The listing builds one solid part. Answer for the finished solid, in the listing's coordinates (mm). A direction names the side the tool comes from. Give positions to 0.01 mm unless a question says otherwise; leave off trailing zeros. Loops run counter-clockwise (first coordinate to the right, second up) from the corner with the lowest first, then second, coordinate; pieces in that order, holes last. Notation, with made-up numbers: (57.5, 76.5) - (101.5, 76.5) arc R30 ccw to (101.5, 99.5) - close; hole circle Ø10 at (-26.75, 42.5). An arc over 180 degrees is marked (long way). Write each question's results on one line, items separated by ' | '.
from build123d import *

# Parameters (mm, degrees)
SKETCH1_R           = 8
SKETCH1_R_2         = 8.25
BOSS_EXTRUDE1_DEPTH = 426


with BuildPart() as part:
    # Sketch1 → Boss-Extrude1 (new body)
    with BuildSketch(Plane.XY):
        with BuildLine():
            Line((-189.997809191, -121.602817484), (-189.997809191, -92.231705942))
            ThreePointArc((-189.997809191, -92.231705942), (-108.380706485, 81.229274354), (-36.431596452, -96.459748112))
            Line((-36.431596452, -96.459748112), (-40.758896177, -121.602817484))
            Line((-40.758896177, -121.602817484), (42.120800042, -121.602817484))
            ThreePointArc((42.120800042, -121.602817484), (-111.259960397, 158.805233349), (-264.640720837, -121.602817484))
            Line((-264.640720837, -121.602817484), (-189.997809191, -121.602817484))
        make_face()
        with Locations((-24.992933093, 62.919265507)):
            Circle(SKETCH1_R, mode=Mode.SUBTRACT)
        with Locations((-197.526987702, 62.919265507)):
            Circle(SKETCH1_R, mode=Mode.SUBTRACT)
        with Locations((-210.852881833, -80.847761798)):
            Circle(SKETCH1_R_2, mode=Mode.SUBTRACT)
        with Locations((-11.667038962, -80.847761798)):
            Circle(SKETCH1_R_2, mode=Mode.SUBTRACT)
    extrude(amount=-BOSS_EXTRUDE1_DEPTH)


solid = part.part
Item 1: Flat-ended cylindrical pins translate along their axes: P1, Ø8, axis at y = 103.5, z = -118.5, coming from the -X side; P2, Ø6, axis at y = -77, z = -167, coming from the -X side; P3, Ø10, axis at y = 96.5, z = -44, coming from the -X side; P4, Ø13, axis at x = -11.67, y = -80.85, coming from the +Z side. Find the tip coordinate at first contact, or state that the pin passes through.
Values found:
P1: stops at x = -245.75 | P2: stops at x = -286.23 | P3: stops at x = -252.64 | P4: passes through
Item 2: For a pull along Y with two mould halves and no side action, classify faces 4 (the face through (-105.802, 158.723, -210.018)), 5 (the face through (-228, -121.603, -210)), 6 (the face through (-17.36, 65.32, -210.02)) as released by +Y, released by -Y, zero draft, split by the parting line, or undercut.
Values found:
face 4: split by the parting line | face 5: released by -Y | face 6: undercut
Item 3: A cutting plane is placed at B-B, the plane z = -70. Determine the outline of the cut face in (x, y), plus the area to 3 significant figures.
Values found:
outline: (-264.64, -121.6) - (-190, -121.6) - (-190, -92.23) arc R104.62 cw (long way) to (-36.43, -96.46) - (-40.76, -121.6) - (42.12, -121.6) arc R182.15 ccw (long way) to start; hole circle Ø16.5 at (-210.85, -80.85); hole circle Ø16 at (-197.53, 62.92); hole circle Ø16 at (-24.99, 62.92); hole circle Ø16.5 at (-11.67, -80.85) | area: 50,300 mm²
Item 4: A cutting plane is placed at A-A, the plane y = -28.5. Determine the outline of the cut face in (x, z).
Values found:
outline: (-293.34, -426) - (-215.75, -426) - (-215.75, 0) - (-293.34, 0) - close; (-6.77, -426) - (70.82, -426) - (70.82, 0) - (-6.77, 0) - close
Item 5: A cutting plane is placed at D-D, the plane x = -92.5. Determine the outline of the cut face in (y, z).
Values found:
outline: (79.57, -426) - (157.84, -426) - (157.84, 0) - (79.57, 0) - close
Item 6: For faces 1 (the face through (-38.565, -108.855, -210.018)), 2 (the face through (-189.998, -107, -210)), 3 (the face through (0, -121.603, -210)), determine the directions among +Z, -Z, +X, -X, +Y, -Y from which every point of the face is accessible in a straight line to the end or side of a thin tool.
Values found:
face 1: +Z, -Z | face 2: +Z, -Z, -Y | face 3: +Z, -Z, +X, -X, -Y
Item 7: Find the intervals of material crossed by line 1 along X through (y, z) = (-77, -179.5); line 2 along Y through (x, z) = (-194, -137.5); line 3 along X through (y, z) = (39, -181), in increasing order. Write a range as [from, to].
Values found:
line 1: x = [-285.33, -218.15], [-203.56, -201.07], [-21.45, -18.96], [-4.37, 62.81] | line 2: y = [-121.6, -87.37], [40.67, 55.74], [70.1, 138.93] | line 3: x = [-282.41, -195.27], [-27.25, 59.89]
Item 8: A cutting plane is placed at C-C, the plane y = 49.5. Determine the outline of the cut face in (x, z), plus the area to 3 significant figures.
Values found:
outline: (-278.21, -426) - (-186.35, -426) - (-186.35, 0) - (-278.21, 0) - close; (-36.17, -426) - (55.69, -426) - (55.69, 0) - (-36.17, 0) - close | area: 78,300 mm²
